Drawing for the job (mm, zero at the part's lowest x, y, z). Round coordinates to 2 decimals unless told otherwise and drop trailing zeros. Write each loop counter-clockwise with the first axis right and the second up, starting at its lowest first coordinate (ties: lowest second). Pieces come first, ordered by that corner, then holes. Notation, with made-up numbers: M 87.5,4 L 124.5,4 A30 ccw 124.5,33 Z; hole C 82.5,5.25 d9. An arc over 180 degrees is marked long. Use a Markdown table: item, result. Add a question column.
1) Wall check: probe 1 along Z at (x, y) = (25.5, 16); probe 2 along X at (y, z) = (15.5, 217); probe 3 along X at (y, z) = (12.75, 305.5). Give the ranges that are in metal, low to high.
2) Slice it at C-C on z = 97.5. Write the cut outline in (x, y).
3) Slice it at A-A on y = 15. Write the cut outline in (x, z).
4) Drop flat-ended pins along their axis: P1, Ø4, axis at x = 6, z = 144, coming from the -Y side; P2, Ø6, axis at x = 11.5, z = 270, coming from the +Y side; P3, Ø3, axis at y = 26.5, z = 114.5, coming from the -X side; P4, Ø6, axis at x = 19.5, y = 19.5, coming from the -Z side. Give the stop position or say it passes through.
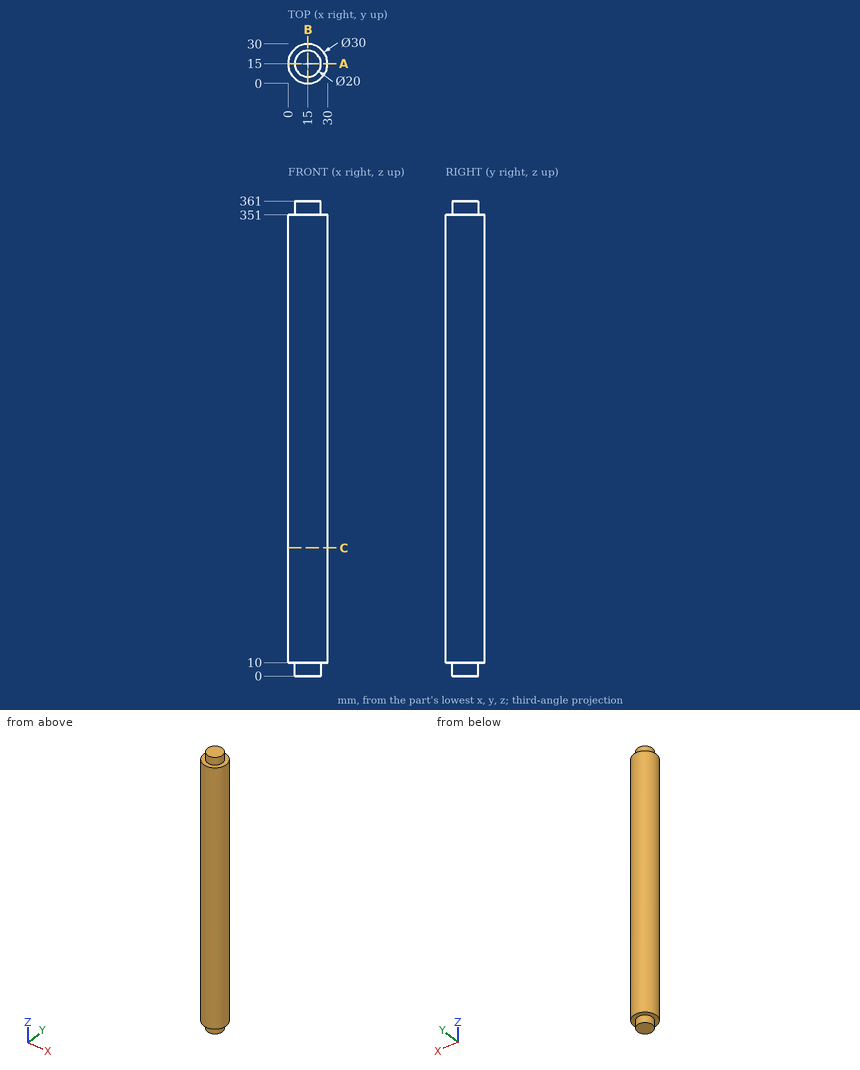
Entries:
| question | item | result |
|---|---|---|
| 1 | probe 1 | z = 10 to 351 |
| 1 | probe 2 | x = 0.01 to 29.99 |
| 1 | probe 3 | x = 0.17 to 29.83 |
| 2 | outline | C 15,15 d30 |
| 3 | outline | M 0,10 L 5,10 L 5,0 L 25,0 L 25,10 L 30,10 L 30,351 L 25,351 L 25,361 L 5,361 L 5,351 L 0,351 Z |
| 4 | P1 | stops at y = 1.73 |
| 4 | P2 | stops at y = 29.99 |
| 4 | P3 | stops at x = 3.82 |
| 4 | P4 | stops at z = 0 |
